The listing builds one solid part. Answer for the finished solid, in the listing's coordinates (mm). Round coordinates to 2 decimals unless told otherwise and drop trailing zeros. Write each loop counter-clockwise with the first axis right and the second up, starting at its lowest first coordinate (ties: lowest second). Pieces come first, ordered by that corner, then holes. Notation, with made-up numbers: M -14.5,29.5 L 42.5,29.5 A33 ccw 42.5,64.5 Z; hole C -30,-26.75 d8. An arc over 180 degrees is marked long. One line per item, written item: value. Start each with the question number.
(1) Given P1, Ø2.5, axis at x = 65.5, y = 24.5, coming from the -Z side; P2, Ø8, axis at x = -27.5, y = 1, coming from the +Z side, each flat-ended and moving along its own axis, determine where each tip first touches the part or whether it passes through.
(2) Section B-B (x = -49.5) is taken. Determine the outline of the cut face in (y, z), plus the area to 3 significant figures.
(3) Consider probe 1 along Y at (x, z) = (65.5, 0.4); probe 2 along Z at (x, y) = (0, 20.5). Determine where each line is inside the solid, lowest interval first.
(4) Section A-A (z = 4.25) is taken. Determine the outline of the cut face in (x, y).
```python
from build123d import *

# Parameters (mm, degrees)
SKETCH1_W           = 140
SKETCH1_H           = 55
SKETCH1_R           = 0.75
BOSS_EXTRUDE1_DEPTH = 1
SKETCH2_W           = 5.209314299
SKETCH2_H           = 7.02492173
BOSS_EXTRUDE2_DEPTH = 5


with BuildPart() as part:
    # Sketch1 → Boss-Extrude1 (new body)
    with BuildSketch(Plane.XY):
        Rectangle(SKETCH1_W, SKETCH1_H)
        with Locations((-65.5, -24.5)):
            Circle(SKETCH1_R, mode=Mode.SUBTRACT)
        with Locations((-65.5, 24.5)):
            Circle(SKETCH1_R, mode=Mode.SUBTRACT)
        with Locations((65.5, 24.5)):
            Circle(SKETCH1_R, mode=Mode.SUBTRACT)
        with Locations((65.5, -24.5)):
            Circle(SKETCH1_R, mode=Mode.SUBTRACT)
    extrude(amount=BOSS_EXTRUDE1_DEPTH)

    # Sketch2 → Boss-Extrude2 (add)
    with BuildSketch(Plane.XY.offset(1)):
        with Locations((67.395342851, 0)):
            Rectangle(SKETCH2_W, SKETCH2_H)
    extrude(amount=BOSS_EXTRUDE2_DEPTH)


solid = part.part
```
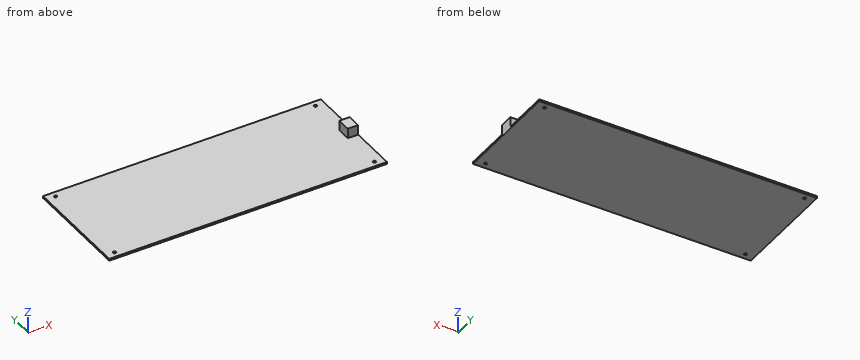
Recorded:
1. P1: stops at z = 0
1. P2: stops at z = 1
2. outline: M -27.5,0 L 27.5,0 L 27.5,1 L -27.5,1 Z
2. area: 55.0 mm2
3. probe 1: y = -27.5 to -25.25, -23.75 to 23.75, 25.25 to 27.5
3. probe 2: z = 0 to 1
4. outline: M 64.79,-3.51 L 70,-3.51 L 70,3.51 L 64.79,3.51 Z
